CAD build for the part. Positions are in the model's coordinates, mm. A direction names the side the tool comes from. Give positions to 0.01 mm unless a question says otherwise; leave off trailing zeros. Loops run counter-clockwise (first coordinate to the right, second up) from the corner with the lowest first, then second, coordinate; pieces in that order, holes last. Notation, with made-up numbers: M -36.75,79 L 6.25,79 A12 cw 6.25,88 Z; hole C 38,82 d5. An arc over 180 degrees is marked long. Answer as CSV lines item,"result".
from build123d import *

# Parameters (mm, degrees)
SKETCH_1_W           = 220
SKETCH_1_H           = 121
EXTRUDE_1_DEPTH      = 7.5
SKETCH_5_W           = 6
SKETCH_5_H           = 8
CUT_EXTRUDE_2_DEPTH  = 165.213275955
SKETCH_9_R           = 22.5
CUT_EXTRUDE_5_DEPTH  = 10
CUT_EXTRUDE_12_DEPTH = 165.213275955
FILLET_1_R           = 5
CHAMFER_1_SIZE       = 0.5
SKETCH_19_R          = 40
CUT_EXTRUDE_13_DEPTH = 159.767912375
CHAMFER_2_SIZE       = 0.5
CHAMFER_4_SIZE       = 0.5


with BuildPart() as part:
    # 草图1 → 凸台-拉伸1 (new, symmetric)
    with BuildSketch(Plane.XY):
        with Locations((0, 60.5)):
            Rectangle(SKETCH_1_W, SKETCH_1_H)
    extrude(amount=EXTRUDE_1_DEPTH, both=True)

    # 草图5 → 切除-拉伸2 (cut, through all)
    with BuildSketch(Plane.XY.offset(7.5)):
        with Locations((-107, 17.5)):
            Rectangle(SKETCH_5_W, SKETCH_5_H)
        with Locations((107, 17.5)):
            Rectangle(SKETCH_5_W, SKETCH_5_H)
    extrude(amount=-CUT_EXTRUDE_2_DEPTH, mode=Mode.SUBTRACT)

    # 草图9 → 切除-拉伸5 (cut)
    with BuildSketch(Plane(origin=(0, 0, -7.5), x_dir=(-1, 0, 0), z_dir=(0, 0, -1))):
        with Locations((0, 66.5)):
            Circle(SKETCH_9_R)
    extrude(amount=-CUT_EXTRUDE_5_DEPTH, mode=Mode.SUBTRACT)

    # 草图4 → 切除-拉伸12 (cut, through all)
    with BuildSketch(Plane.XY.offset(7.5)):
        with BuildLine():
            Line((-94, 66), (-110, 66))
            Line((-110, 66), (-110, 122.2))
            Line((-110, 122.2), (110, 122.2))
            Line((110, 122.2), (110, 66))
            Line((110, 66), (94, 66))
            Line((94, 66), (94, 89.205740869))
            ThreePointArc((94, 89.205740869), (91.081973046, 97.760848899), (83.544303797, 102.749666097))
            ThreePointArc((83.544303797, 102.749666097), (0, 113.5), (-83.544303797, 102.749666097))
            ThreePointArc((-83.544303797, 102.749666097), (-91.081973046, 97.760848899), (-94, 89.205740869))
            Line((-94, 89.205740869), (-94, 66))
        make_face()
    extrude(amount=-CUT_EXTRUDE_12_DEPTH, mode=Mode.SUBTRACT)

    # 圆角1
    fillet_1_edges = [part.edges().sort_by_distance(p)[0] for p in [
        (-110, 66, 0),
        (110, 66, 0),
        (110, 0, 0),
        (-110, 0, 0),
    ]]
    fillet(fillet_1_edges, radius=FILLET_1_R)

    # 倒角1
    chamfer_1_edges = [part.edges().sort_by_distance(p)[0] for p in [
        (-110, 9.25, 7.5),
        (-107, 13.5, 7.5),
        (-104, 17.5, 7.5),
        (-107, 21.5, 7.5),
        (110, 41.25, 7.5),
        (107, 21.5, 7.5),
        (104, 17.5, 7.5),
        (107, 13.5, 7.5),
        (-94, 77.602870434, 7.5),
        (-91.081973046, 97.760848899, 7.5),
        (0, 113.5, 7.5),
        (91.081973046, 97.760848899, 7.5),
        (94, 77.602870434, 7.5),
        (99.5, 66, 7.5),
        (110, 9.25, 7.5),
        (0, 0, 7.5),
        (-99.5, 66, 7.5),
        (-110, 41.25, 7.5),
        (-108.535533906, 64.535533906, 7.5),
        (108.535533906, 64.535533906, 7.5),
        (-108.535533906, 1.464466094, 7.5),
        (108.535533906, 1.464466094, 7.5),
    ]]
    chamfer(chamfer_1_edges, length=CHAMFER_1_SIZE)

    # 草图19 → 切除-拉伸13 (cut, through all)
    with BuildSketch(Plane.XY.offset(7.5)):
        with Locations((0, 55.5)):
            Circle(SKETCH_19_R)
    extrude(amount=-CUT_EXTRUDE_13_DEPTH, mode=Mode.SUBTRACT)

    # 倒角2
    chamfer_2_edges = [part.edges().sort_by_distance(p)[0] for p in [
        (-40, 55.5, 7.5),
    ]]
    chamfer(chamfer_2_edges, length=CHAMFER_2_SIZE)

    # 倒角4
    chamfer_4_edges = [part.edges().sort_by_distance(p)[0] for p in [
        (-110, 13.5, -0.25),
        (-110, 21.5, -0.25),
        (110, 21.5, -0.25),
        (110, 13.5, -0.25),
    ]]
    chamfer(chamfer_4_edges, length=CHAMFER_4_SIZE)


solid = part.part
1) Drill centre lines: line 1 (Y direction, x = 0, z = -2.75); line 2 (X direction, y = 57, z = -4.75); line 3 (Y direction, x = -98, z = -0.25). Where is each one in solid material? Low to high. Write a range as from..to.
Answer below:
line 1,"y = 0..15.5, 95.5..113.5"
line 2,"x = -110..-39.97, 39.97..110"
line 3,"y = 0..66"
2) Band-saw the part on A-A on x = 0. Give the cut face in (y, z), and give its area (3 significant figures).
Answer below:
outline,"M 0,-7.5 L 15.5,-7.5 L 15.5,7 L 15,7.5 L 0.5,7.5 L 0,7 Z; M 95.5,-7.5 L 113.5,-7.5 L 113.5,7 L 113,7.5 L 96,7.5 L 95.5,7 Z"
area,"502 mm^2"
3) Flat gauge pins, fed straight in: pin 1 (6 mm diameter, centred on x = -108, z = -2.5, fed in from +Y); pin 2 (3 mm diameter, centred on x = -107.5, z = 2, fed in from -Y); pin 3 (2 mm diameter, centred on y = 87, z = -0.5, fed in from +X). Where does each tip first touch, or does it go through?
Answer below:
pin 1,"stops at y = 66"
pin 2,"stops at y = 0.1"
pin 3,"stops at x = 94"
4) Band-saw the part on B-B on z = -3.25. Give the cut face in (x, y).
Answer below:
outline,"M -110,5 A5 ccw -105,0 L 105,0 A5 ccw 110,5 L 110,13 L 109.5,13.5 L 104,13.5 L 104,21.5 L 109.5,21.5 L 110,22 L 110,61 A5 ccw 105,66 L 94,66 L 94,89.21 A14 ccw 83.54,102.75 A330 ccw -83.54,102.75 A14 ccw -94,89.21 L -94,66 L -105,66 A5 ccw -110,61 L -110,22 L -109.5,21.5 L -104,21.5 L -104,13.5 L -109.5,13.5 L -110,13 Z; hole C 0,55.5 d80"
5) Which spindle directions (+Z, -Z, +X, -X, +Y, -Y) get a long thin tool onto all of the face, cutting with end or side? Do faces 1 (the face through (104, 17, 0)), 2 (the face through (-1, 0, 0)), 3 (the face through (94, 77, 0)), 4 (the face through (-104, 17, 0)). Say none if no direction does.
Answer below:
face 1,"+Z, -Z, +X"
face 2,"+Z, -Z, +X, -X, -Y"
face 3,"+Z, -Z, +X, +Y"
face 4,"+Z, -Z, -X"
6) Mould opens along X. For faces 5 (the face through (-5.21, 95.16, -0.15)), 6 (the face through (1.182, 113.498, -0.149)), 7 (the face through (-99, 66, 0)), 8 (the face through (-108.246, 64.319, 7.358)) say: +X half, -X half, draft (parallel to the pull), parting line (faces both ways), or undercut.
Answer below:
face 5,"undercut"
face 6,"parting line"
face 7,"draft"
face 8,"-X half"
7) Band-saw the part on C-C on y = 55.5. Give the cut face in (x, z).
Answer below:
outline,"M -110,-7.5 L -40,-7.5 L -40,7 L -40.5,7.5 L -109.5,7.5 L -110,7 Z; M 40,-7.5 L 110,-7.5 L 110,7 L 109.5,7.5 L 40.5,7.5 L 40,7 Z"
